Could you check a few things on this drawing? It's one solid part, dimensions in mm from its lowest x, y, z. Round coordinates to 2 decimals unless told otherwise and drop trailing zeros. Order: outer loops, then holes, each group sorted by start corner. A loop starts at its lowest first (then second) coordinate and runs counter-clockwise, first axis right, second up. Notation, with made-up numbers: (4.25, 38) - (36.25, 38) arc R25 cw to (36.25, 51) - close; hole circle Ø6 at (-9.5, 33). An arc over 180 degrees is marked (long way). Use one line per item in the form item = value.
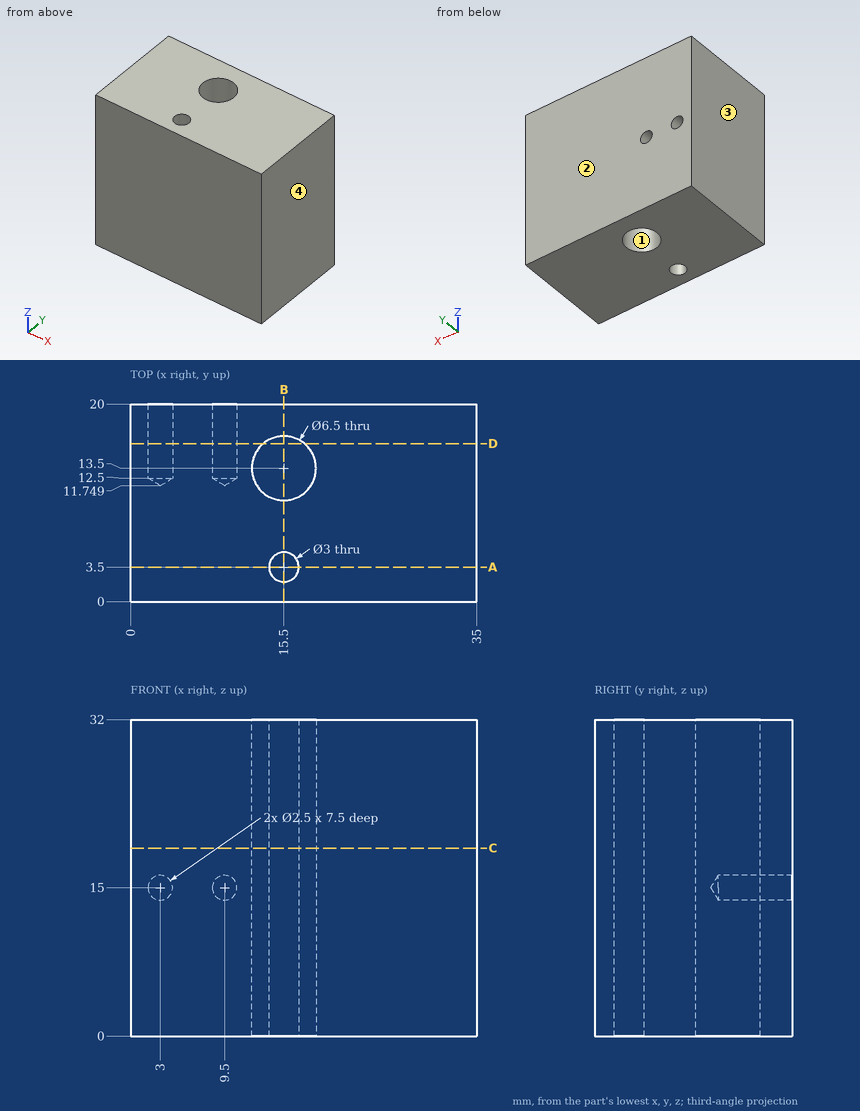
Item 1: Imagine slicing it at D-D on y = 16. Please give me the cut outline in (x, z), plus the area to 3 significant figures.
Found:
outline = (0, 0) - (13.42, 0) - (13.42, 32) - (0, 32) - close; (17.58, 0) - (35, 0) - (35, 32) - (17.58, 32) - close; hole circle Ø2.5 at (3, 15); hole circle Ø2.5 at (9.5, 15)
area = 977 mm2
Item 2: If we mould it in two halves opening along X, with no side actions, what happens to the marked faces 1, 2, 3 and 4? For each: released by +X, released by -X, zero draft, split by the parting line, or undercut.
Found:
face_1 = undercut
face_2 = zero draft
face_3 = released by -X
face_4 = released by +X
Item 3: Imagine slicing it at A-A on y = 3.5. Please give me the cut outline in (x, z), plus the area to 3 significant figures.
Found:
outline = (0, 0) - (14, 0) - (14, 32) - (0, 32) - close; (17, 0) - (35, 0) - (35, 32) - (17, 32) - close
area = 1,020 mm2
Item 4: I need wall thicknesses on L1, parallel to X at y = 18, z = 15; L2, parallel to Y at x = 15.5, z = 17.5; L3, parallel to Z at x = 3, y = 18.25. Which ranges of each line are inside material? Lowest first, please.
Found:
L1 = 0 to 1.75, 4.25 to 8.25, 10.75 to 35
L2 = 0 to 2, 5 to 10.25, 16.75 to 20
L3 = 0 to 13.75, 16.25 to 32
Item 5: Imagine slicing it at C-C on z = 19. Please give me the cut outline in (x, y).
Found:
outline = (0, 0) - (35, 0) - (35, 20) - (0, 20) - close; hole circle Ø6.5 at (15.5, 13.5); hole circle Ø3 at (15.5, 3.5)
Item 6: Will these pins go through, and if not, where does the flat tip stop? P1, Ø4, axis at x = 15.5, y = 13.5, coming from the +Z side; P2, Ø2, axis at x = 9.5, z = 15, coming from the +Y side.
Found:
P1 = through
P2 = 12.35
Item 7: Imagine slicing it at B-B on x = 15.5. Please give me the cut outline in (y, z), plus the area to 3 significant figures.
Found:
outline = (0, 0) - (2, 0) - (2, 32) - (0, 32) - close; (5, 0) - (10.25, 0) - (10.25, 32) - (5, 32) - close; (16.75, 0) - (20, 0) - (20, 32) - (16.75, 32) - close
area = 336 mm2
